```python
from build123d import *

# Parameters (mm, degrees)
SKETCH_1_W                   = 150
SKETCH_1_H                   = 70
EXTRUDE_1_DEPTH              = 10
SKETCH_2_R                   = 10
CUT_EXTRUDE_1_DEPTH          = 55
SKETCH_7_R                   = 5
CUT_EXTRUDE_2_DEPTH          = 20
HOLE_WIZARD_M6_1_D           = 5
HOLE_WIZARD_M6_1_DEPTH       = 13.497848452
HOLE_WIZARD_M6_1_CSINK_D     = 6.05
HOLE_WIZARD_M6_1_CSINK_ANGLE = 90
HOLE_WIZARD_M6_1_TIP         = 1.502151548


with BuildPart() as part:
    # 草图1 → 凸台-拉伸1 (new body)
    with BuildSketch(Plane.XY):
        Rectangle(SKETCH_1_W, SKETCH_1_H)
    extrude(amount=EXTRUDE_1_DEPTH)

    # 草图2 → 切除-拉伸1 (cut)
    with BuildSketch(Plane.XY.offset(10)):
        Circle(SKETCH_2_R)
    extrude(amount=-CUT_EXTRUDE_1_DEPTH, mode=Mode.SUBTRACT)

    # 草图7 → 切除-拉伸2 (cut)
    with BuildSketch(Plane.XY.offset(10)):
        with Locations((-50, 0)):
            Circle(SKETCH_7_R)
        with Locations((50, 0)):
            Circle(SKETCH_7_R)
    extrude(amount=-CUT_EXTRUDE_2_DEPTH, mode=Mode.SUBTRACT)

    # M6 螺纹孔1
    with Locations(Plane.XY.offset(10)):
        with Locations((20, 25), (-20, 25), (-20, -25), (20, -25)):
            CounterSinkHole(HOLE_WIZARD_M6_1_D / 2, HOLE_WIZARD_M6_1_CSINK_D / 2, depth=HOLE_WIZARD_M6_1_DEPTH, counter_sink_angle=HOLE_WIZARD_M6_1_CSINK_ANGLE)
            with Locations((0, 0, -(HOLE_WIZARD_M6_1_DEPTH + HOLE_WIZARD_M6_1_TIP / 2))):  # 118° drill point
                Cone(0, HOLE_WIZARD_M6_1_D / 2, HOLE_WIZARD_M6_1_TIP, mode=Mode.SUBTRACT)


solid = part.part
```
The model under review builds one solid part; all positions refer to its coordinate system, in mm. Round coordinates to 2 decimals unless told otherwise and drop trailing zeros. Order: outer loops, then holes, each group sorted by start corner. A loop starts at its lowest first (then second) coordinate and runs counter-clockwise, first axis right, second up. Notation, with made-up numbers: (18.25, -37.5) -> (33.25, -37.5) arc R5 ccw to (33.25, -32.5) -> close; hole circle Ø5 at (-39, 79.5). An arc over 180 degrees is marked (long way). Use a Markdown table: item, result.
Q1. Clearance check with flat-ended pins moving along their axes: P1, Ø4, axis at x = 20, y = 25, coming from the +Z side; P2, Ø6, axis at x = 20, y = -25, coming from the +Z side (3 decimals); P3, Ø6.5, axis at x = -20, y = -25, coming from the -Z side. State where each tip first meets the part, or that it passes through.
Values:
| item | result |
|---|---|
| P1 | passes through |
| P2 | stops at z = 9.975 |
| P3 | stops at z = 0 |
Q2. We need section A-A on y = 25. Write out the cut boundary in (x, z) (3 decimals).
Values:
| item | result |
|---|---|
| outline | (-75, 0) -> (-22.5, 0) -> (-22.5, 9.475) -> (-23.025, 10) -> (-75, 10) -> close; (-17.5, 0) -> (17.5, 0) -> (17.5, 9.475) -> (16.975, 10) -> (-16.975, 10) -> (-17.5, 9.475) -> close; (22.5, 0) -> (75, 0) -> (75, 10) -> (23.025, 10) -> (22.5, 9.475) -> close |
Q3. Mouldability with a two-part tool opening along X and no side actions: class faces 1 (the flat face through (-75, 0, 5)), 2 (the cylindrical face through (-18.16, 26.69, 4.67)), 3 (the flat face through (75, 0, 5)) as +X half, -X half, draft (parallel to the pull), parting line (faces both ways), or undercut.
Values:
| item | result |
|---|---|
| face 1 | -X half |
| face 2 | undercut |
| face 3 | +X half |
Q4. For line 1 (X direction, y = 25, z = 4); line 2 (Y direction, x = 20, z = 2.5); line 3 (X direction, y = -27, z = 2.5), list the stretches that pass through material, from the lowest coordinate up.
Values:
| item | result |
|---|---|
| line 1 | x = -75 to -22.5, -17.5 to 17.5, 22.5 to 75 |
| line 2 | y = -35 to -27.5, -22.5 to 22.5, 27.5 to 35 |
| line 3 | x = -75 to -21.5, -18.5 to 18.5, 21.5 to 75 |
Q5. We need section D-D on z = 5.25. Write out the cut boundary in (x, y).
Values:
| item | result |
|---|---|
| outline | (-75, -35) -> (75, -35) -> (75, 35) -> (-75, 35) -> close; hole circle Ø10 at (-50, 0); hole circle Ø5 at (-20, -25); hole circle Ø5 at (-20, 25); hole circle Ø20 at (0, 0); hole circle Ø5 at (20, -25); hole circle Ø5 at (20, 25); hole circle Ø10 at (50, 0) |
Q6. We need section C-C on x = -50. Write out the cut boundary in (y, z).
Values:
| item | result |
|---|---|
| outline | (-35, 0) -> (-5, 0) -> (-5, 10) -> (-35, 10) -> close; (5, 0) -> (35, 0) -> (35, 10) -> (5, 10) -> close |
Q7. We need section B-B on x = 20. Write out the cut boundary in (y, z) (3 decimals), then the cut area to 3 significant figures.
Values:
| item | result |
|---|---|
| outline | (-35, 0) -> (-27.5, 0) -> (-27.5, 9.475) -> (-28.025, 10) -> (-35, 10) -> close; (-22.5, 0) -> (22.5, 0) -> (22.5, 9.475) -> (21.975, 10) -> (-21.975, 10) -> (-22.5, 9.475) -> close; (27.5, 0) -> (35, 0) -> (35, 10) -> (28.025, 10) -> (27.5, 9.475) -> close |
| area | 599 mm^2 |
